Geometry check sheet. Reference: the model listing, model coordinates, mm. A direction names the side the tool comes from. Give positions to 0.01 mm unless a question says otherwise; leave off trailing zeros. Write each loop counter-clockwise with the first axis right and the second up, starting at its lowest first coordinate (ties: lowest second). Pieces come first, ordered by that corner, then holes. Notation, with made-up numbers: M 20.25,3 L 50.25,3 A27 cw 50.25,32 Z; hole C 52.25,46.5 d10. An arc over 180 degrees is marked long. Write each question's results on one line, items separated by ' | '.
```python
from build123d import *

# Parameters (mm, degrees)
BASE_PLATE_SKETCH_R     = 6
BASE_PLATE_DEPTH        = 6
UPRIGHT_BORE_SKETCH_R   = 15
UPRIGHT_WITH_BORE_DEPTH = 15
RIB_SKETCH_W            = 12
RIB_SKETCH_H            = 73
RIB_DEPTH               = 70
RIB_WEDGE_CUT_DEPTH     = 70


with BuildPart() as part:
    # Base Plate Sketch → Base Plate (new, symmetric)
    with BuildSketch(Plane(origin=(0, 0, 0), x_dir=(1, 0, 0), z_dir=(0, 1, 0))):
        with BuildLine():
            Line((-20, 25), (-20, 15))
            Line((-20, 15), (-50, 15))
            Line((-50, 15), (-50, -15))
            Line((-50, -15), (-20, -15))
            Line((-20, -15), (-20, -25))
            ThreePointArc((-20, -25), (0, -45), (20, -25))
            Line((20, -25), (20, 25))
            ThreePointArc((20, 25), (0, 45), (-20, 25))
        make_face()
        with Locations(Location((0, 25, 0), (0, 0, 270))):
            Circle(BASE_PLATE_SKETCH_R, mode=Mode.SUBTRACT)
        with Locations(Location((0, -25, 0), (0, 0, 270))):
            Circle(BASE_PLATE_SKETCH_R, mode=Mode.SUBTRACT)
    extrude(amount=BASE_PLATE_DEPTH, both=True)

    # Upright Bore Sketch → Upright with Bore (add, symmetric)
    with BuildSketch(Plane.XY):
        with BuildLine():
            Line((-50, -6), (-75, -6))
            Line((-75, -6), (-75, 44))
            ThreePointArc((-75, 44), (-77.235198346, 50.974858325), (-83.108108108, 55.351351351))
            ThreePointArc((-83.108108108, 55.351351351), (-89.530954843, 99.34333678), (-50, 79))
            Line((-50, 79), (-50, -6))
        make_face()
        with Locations((-75, 79)):
            Circle(UPRIGHT_BORE_SKETCH_R, mode=Mode.SUBTRACT)
    extrude(amount=UPRIGHT_WITH_BORE_DEPTH, both=True)

    # Rib Sketch → Rib (add)
    with BuildSketch(Plane(origin=(-50, 0, 0), x_dir=(0, 0, -1), z_dir=(1, 0, 0))):
        with Locations((1, 42.5)):
            Rectangle(RIB_SKETCH_W, RIB_SKETCH_H)
    extrude(amount=RIB_DEPTH)

    # Rib Wedge Cut Sketch → Rib Wedge Cut (cut)
    with BuildSketch(Plane.XY.offset(5)):
        Polygon((20, 6), (-50, 79), (20, 79), align=None)
    extrude(amount=-RIB_WEDGE_CUT_DEPTH, mode=Mode.SUBTRACT)


solid = part.part
```
Q1. Section check B-B (y = 81.5). Enter the section's corners in (x, z).
Answer key:
outline: M -99.87,-15 L -89.79,-15 L -89.79,15 L -99.87,15 Z; M -60.21,-15 L -50.13,-15 L -50.13,15 L -60.21,15 Z
Q2. Release check for a two-part mould opening along Z. For faces 4 (the face through (-75, 19, 0)), 5 (the face through (0, 0, -31)), 6 (the face through (-59, 50, -15)) record: released by +Z, released by -Z, zero draft, split by the parting line, or undercut.
Answer key:
face 4: zero draft | face 5: undercut | face 6: released by -Z
Q3. Section check D-D (z = -29). Enter the section's corners in (x, y), then the cut area to 3 significant figures.
Answer key:
outline: M -19.6,-6 L -4.47,-6 L -4.47,6 L -19.6,6 Z; M 4.47,-6 L 19.6,-6 L 19.6,6 L 4.47,6 Z | area: 363 mm2
Q4. Depth check by flat-ended pin: P1, Ø20, axis at x = -22, z = 22.5, coming from the +Y side; P2, Ø1.5, axis at y = 34.5, z = -5.5, coming from the +X side; P3, Ø6, axis at x = -32, y = 13, coming from the +Z side. Enter the tip coordinate at first touch or a pass-through.
Answer key:
P1: stops at y = 6 | P2: stops at x = -6.61 | P3: stops at z = 5
Q5. Access from +Z, -Z, +X, -X, +Y, -Y to the whole of each face (thin tool, end or side, straight path). Record for faces 1 (the face through (-59, 50, 15)), 2 (the face through (-8, 6, -22)), 3 (the face through (-23, 34, 5)).
Answer key:
face 1: +Z, -X, +Y, -Y | face 2: -Z, +X, +Y | face 3: +Z, +X, +Y
Q6. Material ranges on probe 1 along X at (y, z) = (2, 25); probe 2 along Z at (x, y) = (-72, 18); probe 3 along Y at (x, z) = (-7.5, 29), recorded low to high. Write a range as [from, to].
Answer key:
probe 1: x = [-20, -6], [6, 20] | probe 2: z = [-15, 15] | probe 3: y = [-6, 6]
Q7. Section check C-C (x = 0). Enter the section's corners in (y, z).
Answer key:
outline: M -6,-45 L 6,-45 L 6,-31 L -6,-31 Z; M -6,-19 L 6,-19 L 6,-7 L 26.86,-7 L 26.86,5 L 6,5 L 6,19 L -6,19 Z; M -6,31 L 6,31 L 6,45 L -6,45 Z
Q8. Section check A-A (z = -2). Enter the section's corners in (x, y).
Answer key:
outline: M -83.11,55.35 A12 cw -75,44 L -75,-6 L 20,-6 L 20,6 L -50,79 A25 ccw long Z; hole C -75,79 d30
